Input: part model. Units: mm. Frame: model coordinates. Face numbers are marked on the shaded views. A direction names the side the tool comes from. Give positions to 0.01 mm unless a question says otherwise; leave off trailing zeros. Write each loop counter-clockwise with the first axis right and the second up, starting at its lowest first coordinate (ties: lowest second). Pieces come first, ordered by that corner, then holes.
```python
from build123d import *

# Parameters (mm, degrees)
CUT_EXTRUDE_1_DEPTH = 2.2
CHAMFER_1_SIZE      = 0.5


with BuildPart() as part:
    # 草图1 → 旋转1 (revolve)
    with BuildSketch(Plane(origin=(0, 0, 0), x_dir=(1, 0, 0), z_dir=(0, 1, 0)), mode=Mode.PRIVATE) as revolve_1_sk:
        Polygon((0, 0), (0, 6), (24, 6), (24, 7.5), (68, 7.5), (68, 10), (233, 10), (233, 7.5), (245, 7.5), (245, 0), align=None)
    revolve(revolve_1_sk.sketch.rotate(Axis((0, 0, 0), (1, 0, 0)), 180), axis=Axis((0, 0, 0), (1, 0, 0)))

    # 草图2 → 切除-拉伸1 (cut)
    with BuildSketch(Plane(origin=(0, -6, 0), x_dir=(-1, 0, 0), z_dir=(0, -1, 0))):
        with BuildLine():
            Line((-21, 2), (-3, 2))
            ThreePointArc((-3, 2), (-1, 0), (-3, -2))
            Line((-3, -2), (-21, -2))
            ThreePointArc((-21, -2), (-23, 0), (-21, 2))
        make_face()
    extrude(amount=-CUT_EXTRUDE_1_DEPTH, mode=Mode.SUBTRACT)

    # 倒角1
    chamfer_1_edges = [part.edges().sort_by_distance(p)[0] for p in [
        (0, 0, -6),
        (245, 0, -7.5),
    ]]
    chamfer(chamfer_1_edges, length=CHAMFER_1_SIZE)


solid = part.part
```
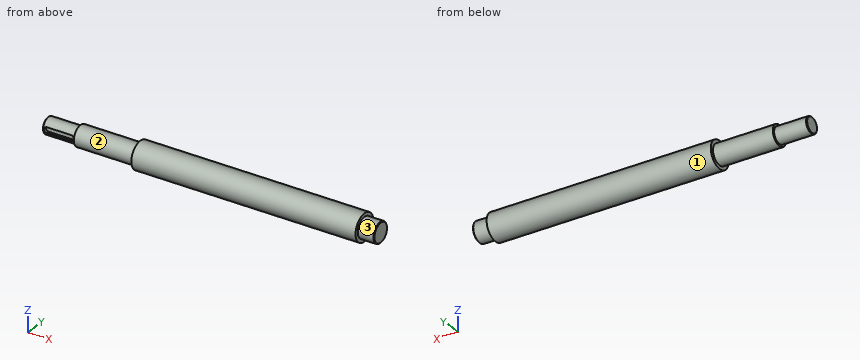
Q1. Section A-A, the plane z = 0. Return the cut outline in (x, y).
Q2. Section C-C, the plane x = 31.5. Return the cut outline in (y, z).
Q3. Section D-D, the plane x = 190.5. Return the cut outline in (y, z).
Q4. Section B-B, the plane y = 0. Return the cut outline in (x, z).
Q5. Access query for the marked faces 1, 2 and 3. Directions: +Z, -Z, +X, -X, +Y, -Y. A direction counts if a zero-diameter tool reaches every point of the face in a straight line with its end or side. Return the directions, or none.
Q6. Pin query (flat end, axial travel): pin 1 (4.5 mm diameter, centred on x = 14.5, z = 0, fed in from -Y); pin 2 (1.5 mm diameter, centred on x = 12, y = -5, fed in from -Z); pin 3 (1 mm diameter, centred on x = 64.5, y = 3, fed in from -Z). Return the tip coordinate at first contact, or that it passes through.
Q7. Material intervals for line 1 along X through (y, z) = (-5.5, 0); line 2 along Y through (x, z) = (217, -0.25); line 3 along Y through (x, z) = (90, -8), sorted ascending.
Solutions:
1. outline: (0, -5.5) - (0.5, -6) - (1, -6) - (1, -3.8) - (23, -3.8) - (23, -6) - (24, -6) - (24, -7.5) - (68, -7.5) - (68, -10) - (233, -10) - (233, -7.5) - (244.5, -7.5) - (245, -7) - (245, 7) - (244.5, 7.5) - (233, 7.5) - (233, 10) - (68, 10) - (68, 7.5) - (24, 7.5) - (24, 6) - (0.5, 6) - (0, 5.5) - close
2. outline: circle Ø15 at (0, 0)
3. outline: circle Ø20 at (0, 0)
4. outline: (0, -5.5) - (0.5, -6) - (24, -6) - (24, -7.5) - (68, -7.5) - (68, -10) - (233, -10) - (233, -7.5) - (244.5, -7.5) - (245, -7) - (245, 7) - (244.5, 7.5) - (233, 7.5) - (233, 10) - (68, 10) - (68, 7.5) - (24, 7.5) - (24, 6) - (0.5, 6) - (0, 5.5) - close
5. face 1: +X, -X
5. face 2: -X
5. face 3: +X
6. pin 1: stops at y = -5.66
6. pin 2: stops at z = -4.24
6. pin 3: stops at z = -7.07
7. line 1: x = 0 to 1, 23 to 245
7. line 2: y = -10 to 10
7. line 3: y = -6 to 6
